Verification items for the finished model (mm, model axes). Coordinates: 2 decimals unless noted, no trailing zeros. Order: outer loops, then holes, each group sorted by start corner. A loop starts at its lowest first (then second) coordinate and runs counter-clockwise, first axis right, second up. Notation, with made-up numbers: (-18.75, 67.5) -> (31.25, 67.5) arc R34 ccw to (31.25, 100.5) -> close; hole circle Ø2 at (30.25, 7.25). An arc over 180 degrees is marked (long way). Write each question's results on one line, items separated by ' | '. Start each with the question number.
(1) Cross-section at A-A on z = 12.5. Give the number of separate pieces and of enclosed holes in the cut face, and give its area (3 significant figures).
(2) Thickness scan on probe 1 along Y at (x, z) = (2185, -14); probe 2 along Y at (x, z) = (2185, 14); probe 3 along Y at (x, z) = (1392, 6.5). Record the ranges inside material, lowest first. Write a range as [from, to].
(3) Go/stop test with flat-tipped pins: pin 1 (9 mm diameter, centred on x = 1725, y = -20, fed in from +Z); pin 2 (6.5 mm diameter, centred on x = 1035.5, y = -16.5, fed in from +Z); pin 3 (1.5 mm diameter, centred on x = 1810.5, z = 4, fed in from +Y); pin 4 (1 mm diameter, centred on x = 1542.5, z = -7.5, fed in from +Y). Record where each tip stops, or that it passes through.
(4) Cross-section at B-B on x = 449. Enter the section's corners in (y, z), and give its area (3 significant figures).
```python
from build123d import *

# Parameters (mm, degrees)
BOSS_EXTRUDE1_DEPTH = 2300
SKETCH2_R           = 5
CUT_EXTRUDE1_DEPTH  = 2301.695547003
SKETCH3_R           = 11
CUT_EXTRUDE2_DEPTH  = 20
LPATTERN1_COUNT     = 10
LPATTERN1_PITCH     = 230


with BuildPart() as part:
    # Sketch1 → Boss-Extrude1 (new body)
    with BuildSketch(Plane(origin=(0, 0, 0), x_dir=(0, 0, -1), z_dir=(1, 0, 0))):
        Polygon((-2.679491924, 40), (-20, 10), (-20, -40), (20, -40), (20, 10), (2.679491924, 40), align=None)
    extrude(amount=BOSS_EXTRUDE1_DEPTH)

    # Sketch2 → Cut-Extrude1 (cut, through all)
    with BuildSketch(Plane.XY.offset(20)):
        with Locations((115, -20)):
            Circle(SKETCH2_R)
    cut_extrude1 = extrude(amount=-CUT_EXTRUDE1_DEPTH, mode=Mode.SUBTRACT)

    # Sketch3 → Cut-Extrude2 (cut)
    with BuildSketch(Plane.XY.offset(20)):
        with Locations((115, -20)):
            Circle(SKETCH3_R)
    cut_extrude2 = extrude(amount=-CUT_EXTRUDE2_DEPTH, mode=Mode.SUBTRACT)

    # LPattern1: Cut-Extrude1, Cut-Extrude2 ×10
    with Locations(*[(i * LPATTERN1_PITCH, 0, 0) for i in range(1, LPATTERN1_COUNT)]):
        add(cut_extrude1, mode=Mode.SUBTRACT)
        add(cut_extrude2, mode=Mode.SUBTRACT)


solid = part.part
```
Results are:
1) separate pieces: 1 | enclosed holes: 10 | area: 141,000 mm2
2) probe 1: y = [-40, -25], [-15, 20.39] | probe 2: y = [-40, -31], [-9, 20.39] | probe 3: y = [-40, 33.38]
3) pin 1: passes through | pin 2: stops at z = 0 | pin 3: stops at y = 39.01 | pin 4: stops at y = 32.52
4) outline: (-40, -20) -> (10, -20) -> (40, -2.68) -> (40, 2.68) -> (10, 20) -> (-40, 20) -> close | area: 2,680 mm2
